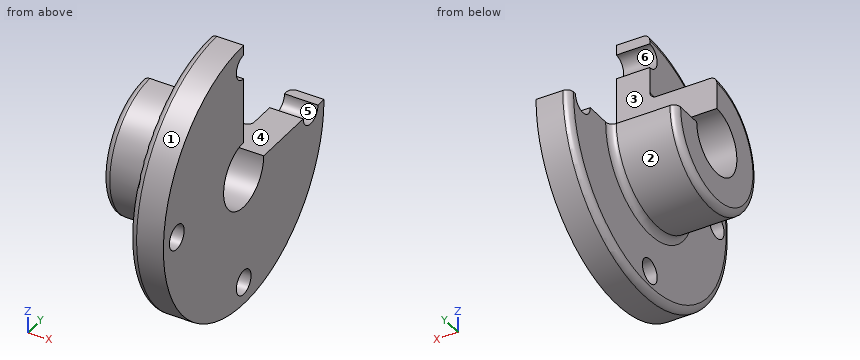
```python
from build123d import *

# Parameters (mm, degrees)
BOLT_HOLES_SKETCH_R = 5.5
BOLT_HOLES_11_DEPTH = 91
EDGE_FILLET_R3_R    = 3
SIDE_CUTOUT_DEPTH   = 97.046863624


with BuildPart() as part:
    # Bed Profile Sketch → Bed Body Revolve (revolve)
    with BuildSketch(Plane.XY, mode=Mode.PRIVATE) as bed_body_revolve_sk:
        Polygon((17.920353982, 15), (17.920353982, 60), (2.920353982, 60), (2.920353982, 30), (-27.079646018, 30), (-27.079646018, 15), align=None)
    revolve(bed_body_revolve_sk.sketch.rotate(Axis((-55.752212389, 0, 0), (1, 0, 0)), 90), axis=Axis((-55.752212389, 0, 0), (1, 0, 0)))

    # Bolt Holes Sketch → Bolt Holes Ø11 (cut, through all)
    with BuildSketch(Plane.ZY.offset(-2.920353982)):
        with Locations((0, 50)):
            Circle(BOLT_HOLES_SKETCH_R)
        with Locations((50, 0)):
            Circle(BOLT_HOLES_SKETCH_R)
        with Locations((0, -50)):
            Circle(BOLT_HOLES_SKETCH_R)
        with Locations((-50, 0)):
            Circle(BOLT_HOLES_SKETCH_R)
    extrude(amount=-BOLT_HOLES_11_DEPTH, mode=Mode.SUBTRACT)

    # Edge Fillet R3
    edge_fillet_r3_edges = [part.edges().sort_by_distance(p)[0] for p in [
        (-27.079646018, 0, -30),
        (2.920353982, 0, -30),
        (2.920353982, 0, -60),
    ]]
    fillet(edge_fillet_r3_edges, radius=EDGE_FILLET_R3_R)

    # Side Cutout Sketch → Side Cutout (cut, through all)
    with BuildSketch(Plane.ZY.offset(27.079646018)):
        with BuildLine():
            Line((0, 77.957463499), (0, 0))
            Line((0, 0), (74.222252728, 0))
            ThreePointArc((74.222252728, 0), (53.256645699, 54.350663604), (0, 77.957463499))
        make_face()
    extrude(amount=-SIDE_CUTOUT_DEPTH, mode=Mode.SUBTRACT)


solid = part.part
```
Check sheet for the modelled part. Datum: model origin and axes. Units: mm. Face numbers are marked on the shaded views. A direction names the side the tool comes from. Coordinates: 2 decimals unless noted, no trailing zeros. Write each loop counter-clockwise with the first axis right and the second up, starting at its lowest first coordinate (ties: lowest second). Pieces come first, ordered by that corner, then holes. Notation, with made-up numbers: M 38,26 L 97,26 A8 cw 97,38 Z; hole C -12,51.25 d1. An arc over 180 degrees is marked long. Write item = value, one per line. Start each with the question number.
1. Thickness scan on probe 1 along Z at (x, y) = (5.5, -2.5); probe 2 along X at (y, z) = (-33, -30); probe 3 along Y at (x, z) = (11.75, -50). Record the ranges inside material, lowest first.
2. Sectioned sample at B-B (z = -4). State how many separate pieces and enclosed holes the cut face has, then the cut area to 3 significant figures.
3. Mould release check, pull along Y, two halves, no side actions. Record for the marked faces 4, 5 and 6: pulls with the +Y half, pulls with the -Y half, needs draft (parallel to the pull), parting line crosses it, or undercut.
4. Tool access check on the marked faces 1, 2 and 3. Record the directions out of +Z, -Z, +X, -X, +Y, -Y that give a thin tool (end or side, any length) a straight path to the whole face; none if there is none.
5. Go/stop test with flat-tipped pins: pin 1 (12 mm diameter, centred on x = 1, y = -36, fed in from -Z); pin 2 (4 mm diameter, centred on x = -7.5, y = -26, fed in from -Z); pin 3 (17.5 mm diameter, centred on y = 0, z = -50, fed in from +X); pin 4 (5 mm diameter, centred on x = 7.5, z = 58.5, fed in from +Y). Record where each tip stops, or that it passes through.
6. Sectioned sample at A-A (x = -2). Record the cut outline in (y, z).
The answers:
q1.probe_1 = -59.92 to -54.9, -45.1 to -14.79, 14.79 to 45.1, 54.9 to 59.92
q1.probe_2 = 2.92 to 17.92
q1.probe_3 = -33.17 to -5.5, 5.5 to 33.17
q2.separate_pieces = 4
q2.enclosed_holes = 0
q2.area = 2,050 mm²
q3.face_4 = needs draft
q3.face_5 = undercut
q3.face_6 = pulls with the +Y half
q4.face_1 = +X, -X
q4.face_2 = -X
q4.face_3 = +Z, +X, -X, +Y
q5.pin_1 = -50.9
q5.pin_2 = -18
q5.pin_3 = 17.92
q5.pin_4 = 0
q6.outline = M 0,15 L 0,30 A30 ccw long 30,0 L 15,0 A15 cw long Z
